```python
from build123d import *

# Parameters (mm, degrees)
SKETCH_1_W      = 100
SKETCH_1_H      = 80
SKETCH_1_R      = 5.5
EXTRUDE_1_DEPTH = 10


with BuildPart() as part:
    # 草图1 → 凸台-拉伸1 (new body)
    with BuildSketch(Plane.XY):
        Rectangle(SKETCH_1_W, SKETCH_1_H)
        with Locations((-35, 30)):
            Circle(SKETCH_1_R, mode=Mode.SUBTRACT)
        with Locations((-35, -30)):
            Circle(SKETCH_1_R, mode=Mode.SUBTRACT)
        with Locations((35, -30)):
            Circle(SKETCH_1_R, mode=Mode.SUBTRACT)
        with Locations((35, 30)):
            Circle(SKETCH_1_R, mode=Mode.SUBTRACT)
    extrude(amount=EXTRUDE_1_DEPTH)


solid = part.part
```
Input: part model. Units: mm. Frame: model coordinates. Coordinates: 2 decimals unless noted, no trailing zeros. Loops run counter-clockwise (first coordinate to the right, second up) from the corner with the lowest first, then second, coordinate; pieces in that order, holes last. Notation, with made-up numbers: (-37.75, -10) - (-20.75, -10) arc R17 cw to (-20.75, 18) - close; hole circle Ø4 at (8, -38). An arc over 180 degrees is marked (long way). Answer in a Markdown table with one row per item.
(1) Material intervals for L1, parallel to Y at x = 35, z = 6.75; L2, parallel to Y at x = 34, z = 2.25; L3, parallel to X at y = 26.5, z = 3.25, sorted ascending. Write a range as from..to.
Model answer:
| item | result |
|---|---|
| L1 | y = -40..-35.5, -24.5..24.5, 35.5..40 |
| L2 | y = -40..-35.41, -24.59..24.59, 35.41..40 |
| L3 | x = -50..-39.24, -30.76..30.76, 39.24..50 |
(2) Cut plane C-C on x = -35. Output: boundary loops of the cut face in (y, z).
Model answer:
| item | result |
|---|---|
| outline | (-40, 0) - (-35.5, 0) - (-35.5, 10) - (-40, 10) - close; (-24.5, 0) - (24.5, 0) - (24.5, 10) - (-24.5, 10) - close; (35.5, 0) - (40, 0) - (40, 10) - (35.5, 10) - close |
(3) Pin query (flat end, axial travel): P1, Ø10, axis at x = -35, y = -30, coming from the -Z side. Return the tip coordinate at first contact, or that it passes through.
Model answer:
| item | result |
|---|---|
| P1 | passes through |
(4) Mould query, pull axis Y, two halves, no side actions, for faces 1 (the face through (29.505, -29.758, 4.93)), 2 (the face through (-1, 1, 0)), 3 (the face through (-1, -40, 5)). Classes: pulls with the +Y half, pulls with the -Y half, needs draft (parallel to the pull), parting line crosses it, or undercut.
Model answer:
| item | result |
|---|---|
| face 1 | undercut |
| face 2 | needs draft |
| face 3 | pulls with the -Y half |
(5) Cut plane B-B on y = -30. Output: boundary loops of the cut face in (x, z), plus the area to 3 significant figures.
Model answer:
| item | result |
|---|---|
| outline | (-50, 0) - (-40.5, 0) - (-40.5, 10) - (-50, 10) - close; (-29.5, 0) - (29.5, 0) - (29.5, 10) - (-29.5, 10) - close; (40.5, 0) - (50, 0) - (50, 10) - (40.5, 10) - close |
| area | 780 mm² |
(6) Cut plane A-A on z = 6.75. Output: boundary loops of the cut face in (x, y).
Model answer:
| item | result |
|---|---|
| outline | (-50, -40) - (50, -40) - (50, 40) - (-50, 40) - close; hole circle Ø11 at (-35, -30); hole circle Ø11 at (-35, 30); hole circle Ø11 at (35, -30); hole circle Ø11 at (35, 30) |
